The drawing under review shows one solid part. Ordinate dimensions are in mm from its lowest x, y, z. Give positions to 0.01 mm unless a question says otherwise; leave off trailing zeros. Order: outer loops, then holes, each group sorted by start corner. A loop starts at its lowest first (then second) coordinate and runs counter-clockwise, first axis right, second up. Notation, with made-up numbers: (-26.75, -1) -> (6.25, -1) arc R23 cw to (6.25, 8) -> close; hole circle Ø11 at (68.25, 52). An arc over 180 degrees is marked (long way). One line per item, written item: value. Start each with the question number.
1) Wall thickness on line 1 along Y through (x, z) = (1, 11.5); line 2 along X through (y, z) = (9.25, 9); line 3 along Y through (x, z) = (8, 20): over which ranges is each line inside the solid? List them lowest first. Write a range as from..to.
2) Consider section C-C (x = 9). State the section outline as (y, z) points.
3) For pin 1 (3.5 mm diameter, centred on x = 8.5, z = 29, fed in from -Y), flat-tipped, find the tip position at first contact; note if it passes through.
4) Consider section B-B (y = 13.25). State the section outline as (x, z) points.
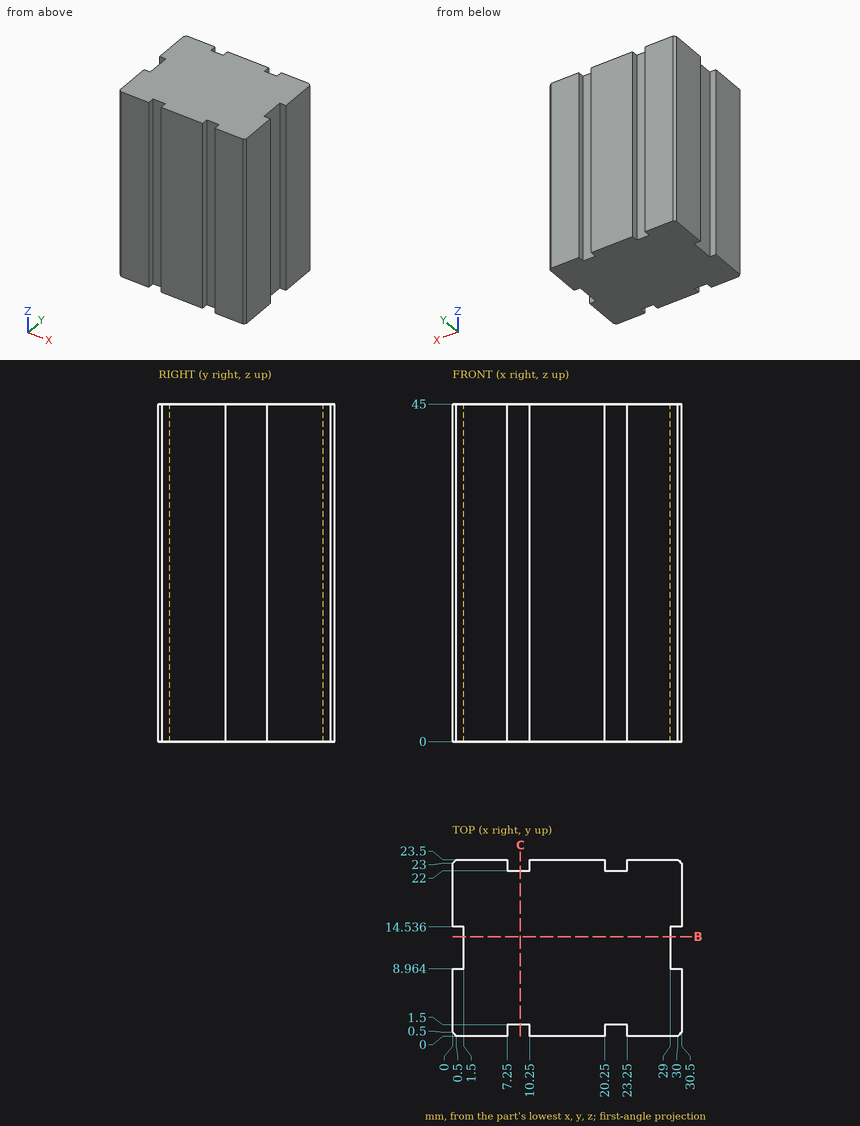
Checked values:
1. line 1: y = 0..8.96, 14.54..23.5
1. line 2: x = 1.5..29
1. line 3: y = 1.5..22
2. outline: (1.5, 0) -> (22, 0) -> (22, 45) -> (1.5, 45) -> close
3. pin 1: stops at y = 0
4. outline: (1.5, 0) -> (29, 0) -> (29, 45) -> (1.5, 45) -> close
